```python
from build123d import *

# Parameters (mm, degrees)
LINK_PROFILES_SKETCH_R   = 15
BASE_LINK_PLATE_DEPTH    = 15
UPPER_START              = 90
UPPER_LINK_PLATE_DEPTH   = 10
LINK_START               = 15
LINK_SLOT_CUT_DEPTH      = 90
SLOT_START               = 80
SKETCH1_7_R              = 15
SLOT_TAB_BOSS_DEPTH      = 10
BRACE_STRUT_A_DEPTH      = 10
BRACE_WEB_A_SKETCH_W     = 25
BRACE_WEB_A_SKETCH_H     = 25
BRACE_WEB_A_DEPTH        = 10
BRACE_STRUT_B_DEPTH      = 10
BRACE_WEB_B_SKETCH_W     = 25
BRACE_WEB_B_SKETCH_H     = 25
BRACE_WEB_B_DEPTH        = 10
SLOTTED_START            = 90
SLOTTED_UPPER_WALL_DEPTH = 50
SIDE_TRIM_CUT_DEPTH      = 150


with BuildPart() as part:
    # Link Profiles Sketch → Base Link Plate (new body)
    with BuildSketch(Plane(origin=(0, 0, 0), x_dir=(1, 0, 0), z_dir=(0, 1, 0))):
        with BuildLine():
            Line((0, 50), (100, 50))
            ThreePointArc((100, 50), (150, 0), (100, -50))
            Line((100, -50), (0, -50))
            ThreePointArc((0, -50), (-50, 0), (0, 50))
        make_face()
        with Locations(Location((0, 0, 0), (0, 0, 270))):
            Circle(LINK_PROFILES_SKETCH_R, mode=Mode.SUBTRACT)
        with Locations(Location((100, 0, 0), (0, 0, 270))):
            Circle(LINK_PROFILES_SKETCH_R, mode=Mode.SUBTRACT)
    extrude(amount=BASE_LINK_PLATE_DEPTH)



with BuildPart() as body_2:
    # Sketch1_5 → Upper Link Plate (new body)
    with BuildSketch(Plane(origin=(0, 0, 0), x_dir=(1, 0, 0), z_dir=(0, 1, 0)).offset(UPPER_START)):
        with BuildLine():
            Line((0, 50), (100, 50))
            ThreePointArc((100, 50), (150, 0), (100, -50))
            Line((100, -50), (0, -50))
            ThreePointArc((0, -50), (-50, 0), (0, 50))
        make_face()
    extrude(amount=-UPPER_LINK_PLATE_DEPTH)

    # Sketch1_6 → Link Slot Cut (cut)
    with BuildSketch(Plane(origin=(0, 0, 0), x_dir=(1, 0, 0), z_dir=(0, 1, 0)).offset(LINK_START)):
        with BuildLine():
            Line((0, 40), (100, 40))
            ThreePointArc((100, 40), (140, 0), (100, -40))
            Line((100, -40), (0, -40))
            ThreePointArc((0, -40), (-40, 0), (0, 40))
        make_face()
    extrude(amount=LINK_SLOT_CUT_DEPTH, mode=Mode.SUBTRACT)


with BuildPart() as body_3:
    # Sketch1_7 → Slot Tab Boss (new body)
    with BuildSketch(Plane(origin=(0, 0, 0), x_dir=(1, 0, 0), z_dir=(0, 1, 0)).offset(SLOT_START)):
        with BuildLine():
            Line((0, 25), (100, 25))
            ThreePointArc((100, 25), (125, 0), (100, -25))
            Line((100, -25), (0, -25))
            ThreePointArc((0, -25), (-25, 0), (0, 25))
        make_face()
        with Locations(Location((0, 0, 0), (0, 0, 270))):
            Circle(SKETCH1_7_R, mode=Mode.SUBTRACT)
        with Locations(Location((100, 0, 0), (0, 0, 270))):
            Circle(SKETCH1_7_R, mode=Mode.SUBTRACT)
    extrude(amount=SLOT_TAB_BOSS_DEPTH)


with BuildPart() as part_1:
    add(part.part)

    add(body_2.part)  # Brace Strut A merges body 2
    # Brace Strut A Sketch → Brace Strut A (add)
    with BuildSketch(Plane.XY.offset(50)):
        Polygon((100, 0), (75, 0), (75, 15), (0, 80), (0, 90), (25, 90), (25, 80), (100, 15), align=None)
    extrude(amount=-BRACE_STRUT_A_DEPTH)


    add(body_3.part)  # Brace Web A merges body 3
    # Brace Web A Sketch → Brace Web A (add)
    with BuildSketch(Plane(origin=(0, 90, 0), x_dir=(1, 0, 0), z_dir=(0, 1, 0))):
        with Locations((12.5, -37.5)):
            Rectangle(BRACE_WEB_A_SKETCH_W, BRACE_WEB_A_SKETCH_H)
    extrude(amount=-BRACE_WEB_A_DEPTH)

    # Brace Strut B Sketch → Brace Strut B (add)
    with BuildSketch(Plane(origin=(0, 0, -50), x_dir=(-1, 0, 0), z_dir=(0, 0, -1))):
        Polygon((0, 0), (-25, 0), (-25, 15), (-100, 80), (-100, 90), (-75, 90), (-75, 80), (0, 15), align=None)
    extrude(amount=-BRACE_STRUT_B_DEPTH)

    # Brace Web B Sketch → Brace Web B (add)
    with BuildSketch(Plane(origin=(0, 90, 0), x_dir=(1, 0, 0), z_dir=(0, 1, 0))):
        with Locations((87.5, 37.5)):
            Rectangle(BRACE_WEB_B_SKETCH_W, BRACE_WEB_B_SKETCH_H)
    extrude(amount=-BRACE_WEB_B_DEPTH)

    # Sketch1_9 → Slotted Upper Wall (add)
    with BuildSketch(Plane(origin=(0, 0, 0), x_dir=(1, 0, 0), z_dir=(0, 1, 0)).offset(SLOTTED_START)):
        with BuildLine():
            Line((0, 50), (100, 50))
            ThreePointArc((100, 50), (150, 0), (100, -50))
            Line((100, -50), (0, -50))
            ThreePointArc((0, -50), (-50, 0), (0, 50))
        make_face()
        with BuildLine():
            Line((0, 40), (100, 40))
            ThreePointArc((100, 40), (140, 0), (100, -40))
            Line((100, -40), (0, -40))
            ThreePointArc((0, -40), (-40, 0), (0, 40))
        make_face(mode=Mode.SUBTRACT)
    extrude(amount=SLOTTED_UPPER_WALL_DEPTH)

    # Side Trim Sketch → Side Trim Cut (cut)
    with BuildSketch(Plane.XY.offset(50)):
        Polygon((150, 90), (-50, 140), (150, 140), align=None)
    extrude(amount=-SIDE_TRIM_CUT_DEPTH, mode=Mode.SUBTRACT)


solid = part_1.part
```
Can you work these out from the model? Positions are in its coordinate system, mm. A direction names the side the tool comes from. Coordinates: 2 decimals unless noted, no trailing zeros. Loops run counter-clockwise (first coordinate to the right, second up) from the corner with the lowest first, then second, coordinate; pieces in that order, holes last.
1) Imagine slicing it at A-A on z = 0. State how many separate pieces and enclosed holes the cut face has, plus the area to 3 significant figures.
2) For pin 1 (11 mm diameter, centred on y = 87, z = -36, fed in from +X); pin 2 (1.5 mm diameter, centred on x = 120, z = 22.5, fed in from +Y); pin 3 (5 mm diameter, centred on y = 114, z = 13, fed in from +X), each with a flat end and sliding along its axis, tell me the tip position at first contact or that it passes through.
3) Imagine slicing it at C-C on y = 114.5. List the corners of the cut face in (x, z) for me.
4) Imagine slicing it at B-B on x = 43. List the corners of the cut face in (y, z) for me, plus the area to 3 significant figures.
5) Which directions (+Z, -Z, +X, -X, +Y, -Y) give clear straight access to the entire face, cutting with the end or side of a thin tool? Please do faces 1 (the cylindrical face through (0.66, 84.93, -14.985)), 2 (the flat face through (50, 50, 40)), 3 (the cylindrical face through (149.988, 88.592, -1.099)), 4 (the flat face through (49, 90, -1)), 5 (the flat face through (61.98, 47.05, -45.07)).
6) I need wall thicknesses on probe 1 along X at (y, z) = (87, 0); probe 2 along Y at (x, z) = (13, -23); probe 3 along Z at (x, y) = (30, 75). Which ranges of each line are inside material? Lowest first, please.
7) Imagine slicing it at D-D on y = 27. List the corners of the cut face in (x, z) for me.
8) Thinking about a two-plate mould opening in X: for faces 6 (the cylindrical face through (-49.988, 7.395, 1.099)), 7 (the flat face through (25, 85, 33)), 8 (the flat face through (50, 115, 41)), 9 (the cylindrical face through (-24.994, 84.93, 0.55)), which applies, pulls with the +X half, pulls with the -X half, needs draft (parallel to the pull), parting line crosses it, or undercut?
Completed:
1. separate pieces: 8
1. enclosed holes: 0
1. area: 3,700 mm2
2. pin 1: stops at x = 139.62
2. pin 2: stops at y = 15
2. pin 3: stops at x = -36.87
3. outline: (0, -50) - (52, -50) - (52, -40) - (0, -40) arc R40 cw to (0, 40) - (52, 40) - (52, 50) - (0, 50) arc R50 ccw to start
4. outline: (0, -50) - (15, -50) - (15, 50) - (0, 50) - close; (30.6, -50) - (52.27, -50) - (52.27, -40) - (30.6, -40) - close; (42.73, 40) - (64.4, 40) - (64.4, 50) - (42.73, 50) - close; (80, -50) - (116.75, -50) - (116.75, -40) - (80, -40) - close; (80, -25) - (90, -25) - (90, 25) - (80, 25) - close; (80, 40) - (116.75, 40) - (116.75, 50) - (80, 50) - close
4. area: 3,170 mm2
5. face 1: +Y, -Y
5. face 2: +X, -X
5. face 3: +X, +Y, -Y
5. face 4: +Y
5. face 5: -Z, +X
6. probe 1: x = -50 to -40, -25 to -15, 15 to 85, 115 to 125, 140 to 150
6. probe 2: y = 0 to 15, 80 to 90
6. probe 3: z = 40 to 50
7. outline: (13.85, -50) - (38.85, -50) - (38.85, -40) - (13.85, -40) - close; (61.15, 40) - (86.15, 40) - (86.15, 50) - (61.15, 50) - close
8. face 6: pulls with the -X half
8. face 7: undercut
8. face 8: pulls with the +X half
8. face 9: undercut
